```python
from build123d import *

# Parameters (mm, degrees)
SKETCH_2_W     = 1.5
SKETCH_2_H     = 4.230303993
CHAMFER_1_SIZE = 1


with BuildPart() as part:
    # 草图1 → 旋转1 (revolve)
    with BuildSketch(Plane(origin=(0, 0, 0), x_dir=(-1, 0, 0), z_dir=(0, 0, -1)), mode=Mode.PRIVATE) as revolve_1_sk:
        Polygon((-17.5, 5), (-17.5, 0), (17.5, 0), (17.5, 5), (-13, 5), (-13, 4), (-14.05, 4), (-14.05, 5), align=None)
    revolve(revolve_1_sk.sketch.rotate(Axis((17.5, 0, 0), (-1, 0, 0)), 270), axis=Axis((17.5, 0, 0), (-1, 0, 0)))

    # 草图2 → 旋转2 (revolve)
    with BuildSketch(Plane(origin=(-13.5, 0, 0), x_dir=(0, 0, -1), z_dir=(1, 0, 0))):
        with Locations((0.75, -6.884848004)):
            Rectangle(SKETCH_2_W, SKETCH_2_H)
    revolve(axis=Axis((-13.5, -4.769696007, 0), (0, -1, 0)))

    # 倒角1
    chamfer_1_edges = [part.edges().sort_by_distance(p)[0] for p in [
        (17.5, 0, -5),
        (-17.5, 0, -5),
    ]]
    chamfer(chamfer_1_edges, length=CHAMFER_1_SIZE)


solid = part.part
```
Geometry check sheet. Reference: the model listing, model coordinates, mm. Give positions to 0.01 mm unless a question says otherwise; leave off trailing zeros. Loops run counter-clockwise (first coordinate to the right, second up) from the corner with the lowest first, then second, coordinate; pieces in that order, holes last. Notation, with made-up numbers: M 47,85.25 L 80,85.25 A12 cw 80,92.25 Z; hole C 66.5,9 d4. An arc over 180 degrees is marked long. Answer as CSV lines item,"result".
Item 1: Cross-section at D-D on x = 8. Record the cut outline in (y, z), and give its area (3 significant figures).
Values:
outline,"C 0,0 d10"
area,"78.5 mm²"
Item 2: Cross-section at A-A on z = 0. Record the cut outline in (x, y).
Values:
outline,"M -17.5,-4 L -16.5,-5 L -15,-5 L -15,-9 L -12,-9 L -12,-5 L 13,-5 L 13,-4 L 14.05,-4 L 14.05,-5 L 16.5,-5 L 17.5,-4 L 17.5,4 L 16.5,5 L 14.05,5 L 14.05,4 L 13,4 L 13,5 L -16.5,5 L -17.5,4 Z"
Item 3: Cross-section at B-B on x = -13.5. Record the cut outline in (y, z).
Values:
outline,"M -9,-1.5 L -4.77,-1.5 A5 ccw long -4.77,1.5 L -9,1.5 Z"
Item 4: Release check for a two-part mould opening along X. For faces 1 (the flat face through (-17.5, 0, 0)), 2 (the cylindrical face through (13.532, -3.905, -0.867)), 3 (the flat face through (17.5, 0, 0)), 4 (the flat face through (-13, -9, 0)) record: pulls with the +X half, pulls with the -X half, needs draft (parallel to the pull), parting line crosses it, or undercut.
Values:
face 1,"pulls with the -X half"
face 2,"undercut"
face 3,"pulls with the +X half"
face 4,"needs draft"
Item 5: Depth check by flat-ended pin: P1, Ø8, axis at x = -6.5, y = -7.5, coming from the -Z side; P2, Ø4, axis at y = -7, z = 2.5, coming from the +X side; P3, Ø1, axis at x = -11.5, z = -3, coming from the +Y side. Enter the tip coordinate at first touch or a pass-through.
Values:
P1,"stops at z = -3.57"
P2,"stops at x = -12.09"
P3,"stops at y = 4.33"
Item 6: Cross-section at C-C on y = -5.5. Record the cut outline in (x, z), and give its area (3 significant figures).
Values:
outline,"C -13.5,0 d3"
area,"7.07 mm²"
Item 7: Material ranges on line 1 (X direction, y = -4.25, z = -2); line 2 (X direction, y = 4.5, z = -1); line 3 (X direction, y = -5.5, z = 0), recorded low to high.
Values:
line 1,"x = -16.8 to 13, 14.05 to 16.8"
line 2,"x = -16.89 to 13, 14.05 to 16.89"
line 3,"x = -15 to -12"
